Check sheet for the modelled part. Datum: model origin and axes. Units: mm. Face numbers are marked on the shaded views. A direction names the side the tool comes from. Give positions to 0.01 mm unless a question says otherwise; leave off trailing zeros. Loops run counter-clockwise (first coordinate to the right, second up) from the corner with the lowest first, then second, coordinate; pieces in that order, holes last. Notation, with made-up numbers: (42.5, 10.25) - (57.5, 10.25) arc R15 cw to (57.5, 31.25) - close; hole circle Ø5 at (69, 16.5). An arc over 180 degrees is marked (long way). Answer in a Markdown table with one row per item. Add a question column.
(1) Set-up check for the marked faces 1 and 2: record each of +Z, -Z, +X, -X, +Y, -Y from which the full face is reachable in a straight line by a thin tool's end or side.
(2) Thickness scan on L1, parallel to Y at x = 30, z = 0; L2, parallel to Z at x = -33.5, y = 3; L3, parallel to Z at x = -10, y = 6.5. Record the ranges inside material, lowest first.
(3) Sectioned sample at C-C on x = -7. Enter the section's corners in (y, z).
(4) Draft check along Z on the marked faces 3, 4 and 5. Enter one of: released by +Z, released by -Z, zero draft, split by the parting line, or undercut.
(5) Go/stop test with flat-tipped pins: P1, Ø13, axis at y = -60.5, z = 0, coming from the -X side; P2, Ø6, axis at x = 11.5, z = -50, coming from the -Y side; P3, Ø2.5, axis at y = -1, z = 60.5, coming from the -X side; P4, Ø2, axis at x = 11.5, z = -28.5, coming from the +Y side. Record where each tip stops, or that it passes through.
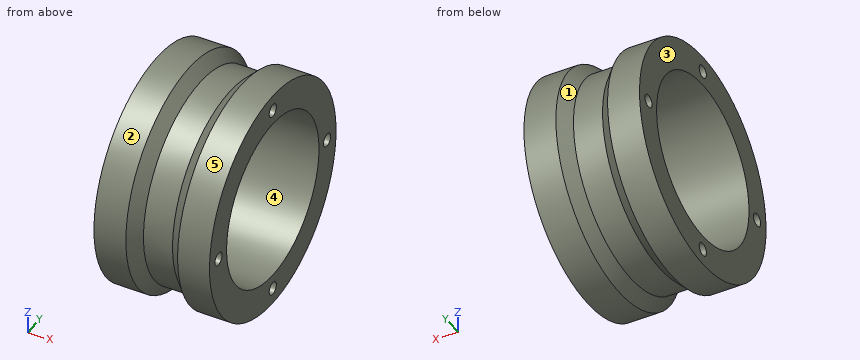
from build123d import *

# Parameters (mm, degrees)
SKETCH4_R          = 4
CUT_EXTRUDE1_DEPTH = 13
CUT_EXTRUDE2_START = -13
SKETCH5_R          = 4
CUT_EXTRUDE2_DEPTH = 13


with BuildPart() as part:
    # Sketch2 → Revolve1 (revolve)
    with BuildSketch(Plane.XY, mode=Mode.PRIVATE) as revolve1_sk:
        Polygon((-37.225396825, 70.5), (-37.225396825, 51.5), (34.274603175, 51.5), (34.274603175, 70.5), (14.524603175, 70.5), (7.524603175, 63.5), (-10.475396825, 63.5), (-17.475396825, 70.5), align=None)
    revolve(revolve1_sk.sketch.rotate(Axis((-86.707936508, 0, 0), (1, 0, 0)), 90), axis=Axis((-86.707936508, 0, 0), (1, 0, 0)))

    # Sketch4 → Cut-Extrude1 (cut)
    with BuildSketch(Plane.ZY.offset(37.225396825)):
        with Locations((0, -60.5)):
            Circle(SKETCH4_R)
        with Locations((-60.5, 0)):
            Circle(SKETCH4_R)
        with Locations((0, 60.5)):
            Circle(SKETCH4_R)
        with Locations((60.5, 0)):
            Circle(SKETCH4_R)
    extrude(amount=-CUT_EXTRUDE1_DEPTH, mode=Mode.SUBTRACT)

    # Sketch5 → Cut-Extrude2 (cut)
    with BuildSketch(Plane(origin=(34.274603175, 0, 0), x_dir=(0, 0, -1), z_dir=(1, 0, 0)).offset(CUT_EXTRUDE2_START)):
        with Locations(Location((0, -60.5, 0), (0, 0, 180))):
            Circle(SKETCH5_R)
        with Locations(Location((-60.5, 0, 0), (0, 0, 180))):
            Circle(SKETCH5_R)
        with Locations(Location((0, 60.5, 0), (0, 0, 180))):
            Circle(SKETCH5_R)
        with Locations(Location((60.5, 0, 0), (0, 0, 180))):
            Circle(SKETCH5_R)
    extrude(amount=CUT_EXTRUDE2_DEPTH, mode=Mode.SUBTRACT)


solid = part.part
Reply:
| question | item | result |
|---|---|---|
| 1 | face 1 | none |
| 1 | face 2 | +X, -X |
| 2 | L1 | -70.5 to -64.5, -56.5 to -51.5, 51.5 to 56.5, 64.5 to 70.5 |
| 2 | L2 | -70.44 to -63.15, -57.85 to -51.41, 51.41 to 57.85, 63.15 to 70.44 |
| 2 | L3 | -63.17 to -51.09, 51.09 to 63.17 |
| 3 | outline | circle Ø127 at (0, 0); hole circle Ø103 at (0, 0) |
| 4 | face 3 | zero draft |
| 4 | face 4 | undercut |
| 4 | face 5 | split by the parting line |
| 5 | P1 | x = -37.23 |
| 5 | P2 | y = -50.59 |
| 5 | P3 | x = -24.23 |
| 5 | P4 | y = 62.35 |
